Design review of the part built by this model. Coordinates are the model's own, in mm. Face numbers are marked on the shaded views. A direction names the side the tool comes from. Round coordinates to 2 decimals unless told otherwise and drop trailing zeros. Order: outer loops, then holes, each group sorted by start corner. A loop starts at its lowest first (then second) coordinate and runs counter-clockwise, first axis right, second up. Notation, with made-up numbers: (14.25, -35) - (39.25, -35) arc R18 ccw to (39.25, -6) - close; hole circle Ø8 at (7, 61). An arc over 180 degrees is marked (long way). Answer as a JSON object with one key per item and string values. Group by question number.
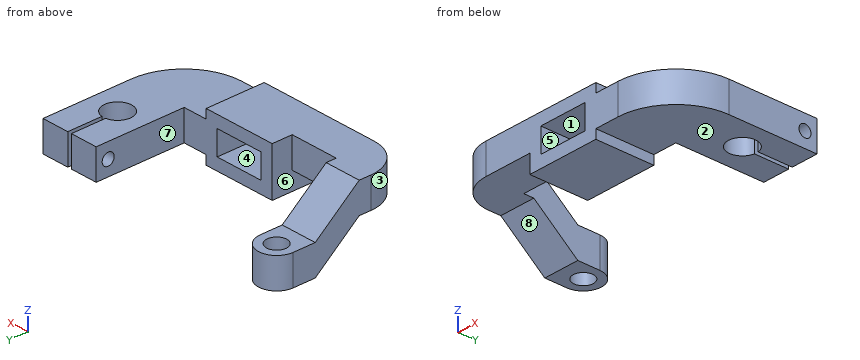
from build123d import *

# Parameters (mm, degrees)
Z_PROFILE_PLATE_DEPTH       = 15
ARM_EXTENSION_BOSS_DEPTH    = 24
CLAMP_START                 = -4.5
CLAMP_HUB_BOSS_DEPTH        = 15
CENTER_BLOCK_DEPTH          = 18
PIVOT_START                 = -1.5
PIVOT_LUG_DEPTH             = 7.5
PIVOT_HOLE_SKETCH_R         = 5
PIVOT_HOLE_10_DEPTH         = 15
RECTANGULAR_POCKET_SKETCH_W = 24
RECTANGULAR_POCKET_SKETCH_H = 12
RECTANGULAR_POCKET_DEPTH    = 116.004347744
CLAMP_SLOT_DEPTH            = 15
CLAMP_SCREW_HOLE_SKETCH_R   = 3
CLAMP_SCREW_HOLE_6_DEPTH    = 121.490663539


with BuildPart() as part:
    # Z Profile Sketch → Z Profile Plate (new body)
    with BuildSketch(Plane.XY):
        with BuildLine():
            ThreePointArc((-18, 18), (-12.727922061, 5.272077939), (0, 0))
            Line((0, 0), (24, 0))
            Line((24, 0), (24, 19))
            Line((24, 19), (0, 19))
            Line((0, 19), (0, 24))
            Line((0, 24), (-16.970562748, 24))
            Line((-16.970562748, 24), (-18, 24))
            Line((-18, 24), (-18, 18))
        make_face()
    extrude(amount=-Z_PROFILE_PLATE_DEPTH)

    # Sketch1_6 → Arm Extension Boss (add)
    with BuildSketch(Plane.XY):
        Polygon((24, 19), (24, 0), (60, 0), (60, 29), (24, 29), align=None)
    extrude(amount=-ARM_EXTENSION_BOSS_DEPTH)

    # Sketch1_7 → Clamp Hub Boss (add)
    with BuildSketch(Plane.XY.offset(CLAMP_START)):
        with BuildLine():
            Line((60, 0), (72, 0))
            ThreePointArc((72, 0), (92.506096654, 8.493903346), (101, 29))
            Line((101, 29), (101, 73))
            Line((101, 73), (72, 73))
            Line((72, 73), (72, 29))
            Line((72, 29), (60, 29))
            Line((60, 29), (60, 0))
        make_face()
    extrude(amount=-CLAMP_HUB_BOSS_DEPTH)

    # Center Block Sketch → Center Block (add)
    with BuildSketch(Plane.ZY.offset(18)):
        Polygon((-33, 46), (-15, 24), (0, 24), (-18, 46), align=None)
    extrude(amount=-CENTER_BLOCK_DEPTH)

    # Pivot Lug Sketch → Pivot Lug (add, symmetric)
    with BuildSketch(Plane.XY.offset(-24).offset(PIVOT_START)):
        with BuildLine():
            Line((-18, 57), (-18, 46))
            Line((-18, 46), (0, 46))
            Line((0, 46), (0, 57))
            ThreePointArc((0, 57), (-9, 66), (-18, 57))
        make_face()
    extrude(amount=PIVOT_LUG_DEPTH, both=True)

    # Pivot Hole Sketch → Pivot Hole _10 (cut)
    with BuildSketch(Plane.XY.offset(-18)):
        with Locations((-9, 57)):
            Circle(PIVOT_HOLE_SKETCH_R)
    extrude(amount=-PIVOT_HOLE_10_DEPTH, mode=Mode.SUBTRACT)

    # Rectangular Pocket Sketch → Rectangular Pocket (cut, through all)
    with BuildSketch(Plane(origin=(0, 29, 0), x_dir=(1, 0, 0), z_dir=(0, 1, 0))):
        with Locations((42, 12)):
            Rectangle(RECTANGULAR_POCKET_SKETCH_W, RECTANGULAR_POCKET_SKETCH_H)
    extrude(amount=-RECTANGULAR_POCKET_DEPTH, mode=Mode.SUBTRACT)

    # Clamp Slot Sketch → Clamp Slot (cut)
    with BuildSketch(Plane.XY.offset(-4.5)):
        with BuildLine():
            Line((87.5, 55.92820323), (87.5, 73))
            Line((87.5, 73), (85.5, 73))
            Line((85.5, 73), (85.5, 55.92820323))
            ThreePointArc((85.5, 55.92820323), (86.5, 42), (87.5, 55.92820323))
        make_face()
    extrude(amount=-CLAMP_SLOT_DEPTH, mode=Mode.SUBTRACT)

    # Clamp Screw Hole Sketch → Clamp Screw Hole _6 (cut, through all)
    with BuildSketch(Plane.ZY.offset(-72)):
        with Locations((-12, 67)):
            Circle(CLAMP_SCREW_HOLE_SKETCH_R)
    extrude(amount=-CLAMP_SCREW_HOLE_6_DEPTH, mode=Mode.SUBTRACT)


solid = part.part
1. To check wall thickness, follow line 1 (Z direction, x = -5.5, y = 3.5); line 2 (Z direction, x = 77.5, y = 17); line 3 (Y direction, x = 64.5, z = -9.5). State the ranges of each line that lie inside material, in increasing order. Write a range as from..to.
2. Tool access review of the marked faces 5, 6, 7 and 8: name each direction out of +Z, -Z, +X, -X, +Y, -Y from which nothing blocks a thin tool from reaching the whole face with its end or side.
3. Take a section at C-C, the plane y = 39. Give the boundary of the cut face in (x, z), then the cut area to 3 significant figures.
4. Clearance check with flat-ended pins moving along their axes: P1, Ø9.5, axis at y = 67, z = -12, coming from the +X side; P2, Ø22.5, axis at x = 86.5, y = 49, coming from the +Z side; P3, Ø23, axis at x = 40, y = 17, coming from the -Z side; P4, Ø7, axis at x = 11, y = 16, coming from the -Z side. State where each tip first meets the part, or that it passes through.
5. Mouldability with a two-part tool opening along Z and no side actions: class the marked faces 1, 2, 3 and 4 as pulls with the +Z half, pulls with the -Z half, needs draft (parallel to the pull), parting line crosses it, or undercut.
6. Take a section at D-D, the plane z = -12. Give the boundary of the cut face in (x, y), then the cut area to 4 significant figures.
7. Take a section at A-A, the plane y = 49. Give the boundary of the cut face in (x, z).
8. Take a section at B-B, the plane x = 33. Give the boundary of the cut face in (y, z).
Response values:
{
 "1": {"line 1": "-15..0", "line 2": "-19.5..-4.5", "line 3": "0..29"},
 "2": {"face 5": "+Y, -Y", "face 6": "-Z, +Y", "face 7": "+Z, -Z, +Y", "face 8": "-Z, -X, -Y"},
 "3": {"outline": "(-18, -27.27) - (0, -27.27) - (0, -12.27) - (-18, -12.27) - close; (72, -19.5) - (101, -19.5) - (101, -4.5) - (72, -4.5) - close", "area": "705 mm2"},
 "4": {"P1": "x = 101", "P2": "z = -4.5", "P3": "z = -24", "P4": "z = -15"},
 "5": {"face 1": "undercut", "face 2": "pulls with the -Z half", "face 3": "needs draft", "face 4": "undercut"},
 "6": {"outline": "(-18, 18) arc R18 ccw to (0, 0) - (30, 0) - (30, 29) - (24, 29) - (24, 19) - (0, 19) - (0, 38.67) - (-18, 38.67) - close; (54, 0) - (72, 0) arc R29 ccw to (101, 29) - (101, 64) - (87.5, 64) - (87.5, 55.93) arc R7 cw (long way) to (85.5, 55.93) - (85.5, 64) - (72, 64) - (72, 29) - (54, 29) - close; (72, 70) - (85.5, 70) - (85.5, 73) - (72, 73) - close; (87.5, 70) - (101, 70) - (101, 73) - (87.5, 73) - close", "area": "3,365 mm2"},
 "7": {"outline": "(-18, -33) - (0, -33) - (0, -18) - (-18, -18) - close; (72, -19.5) - (79.5, -19.5) - (79.5, -4.5) - (72, -4.5) - close; (93.5, -19.5) - (101, -19.5) - (101, -4.5) - (93.5, -4.5) - close"},
 "8": {"outline": "(0, -24) - (29, -24) - (29, -18) - (0, -18) - close; (0, -6) - (29, -6) - (29, 0) - (0, 0) - close"}
}
